Read the model definition and answer for the solid it produces. Units are mm, in the model's axes. Face numbers are marked on the shaded views. Coordinates: 2 decimals unless noted, no trailing zeros. One line per item, written item: value. Start each with the question number.
1. For a pull along X with two mould halves and no side action, classify the marked faces 1 and 2 as pulls with the +X half, pulls with the -X half, needs draft (parallel to the pull), parting line crosses it, or undercut.
2. Given P1, Ø1, axis at x = -81.5, y = 5.5, coming from the -Z side; P2, Ø5, axis at x = -4.5, y = 31, coming from the +Z side; P3, Ø4, axis at y = 23, z = 21.5, coming from the -X side; P4, Ø15.5, axis at x = -4.5, z = -5, coming from the +Y side, each flat-ended and moving along its own axis, determine where each tip first touches the part or whether it passes through.
3. Consider line 1 along X through (y, z) = (19.5, 0); line 2 along Z through (x, y) = (1.5, 19); line 3 along Y through (x, z) = (90.5, 48.5). Determine where each line is inside the solid, lowest interval first.
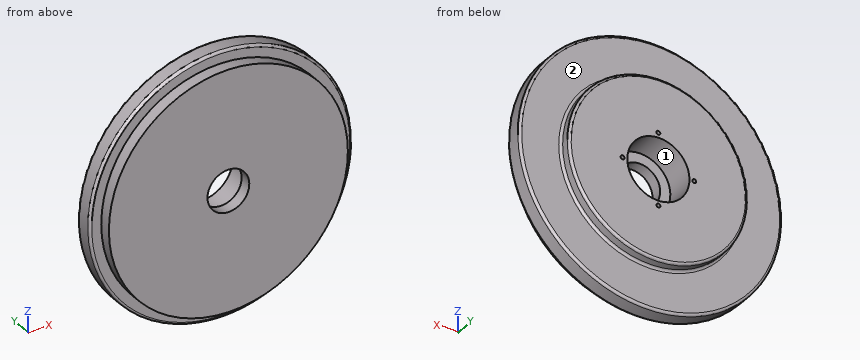
```python
from build123d import *

# Parameters (mm, degrees)
SKETCH1_R           = 100
BOSS_EXTRUDE1_DEPTH = 10
SKETCH2_R           = 110
BOSS_EXTRUDE2_DEPTH = 15
SKETCH3_R           = 75
BOSS_EXTRUDE3_DEPTH = 10
FILLET1_R           = 2
SKETCH4_R           = 26
CUT_EXTRUDE1_DEPTH  = 25
SKETCH5_R           = 17.5
CUT_EXTRUDE2_DEPTH  = 158.559512566
CIRPATTERN1_COUNT   = 4
FILLET2_R           = 2


with BuildPart() as part:
    # Sketch1 → Boss-Extrude1 (new body)
    with BuildSketch(Plane(origin=(0, 0, 0), x_dir=(1, 0, 0), z_dir=(0, 1, 0))):
        with Locations(Location((0, 0, 0), (0, 0, 270))):
            Circle(SKETCH1_R)
    extrude(amount=BOSS_EXTRUDE1_DEPTH)

    # Sketch2 → Boss-Extrude2 (add)
    with BuildSketch(Plane(origin=(0, 10, 0), x_dir=(1, 0, 0), z_dir=(0, 1, 0))):
        with Locations(Location((0, 0, 0), (0, 0, 270))):
            Circle(SKETCH2_R)
    extrude(amount=BOSS_EXTRUDE2_DEPTH)

    # Sketch3 → Boss-Extrude3 (add)
    with BuildSketch(Plane(origin=(0, 25, 0), x_dir=(1, 0, 0), z_dir=(0, 1, 0))):
        with Locations(Location((0, 0, 0), (0, 0, 270))):
            Circle(SKETCH3_R)
    extrude(amount=BOSS_EXTRUDE3_DEPTH)

    # Fillet1
    fillet1_edges = [part.edges().sort_by_distance(p)[0] for p in [
        (0, 25, -75),
        (0, 35, -75),
    ]]
    fillet(fillet1_edges, radius=FILLET1_R)

    # Sketch4 → Cut-Extrude1 (cut)
    with BuildSketch(Plane(origin=(0, 35, 0), x_dir=(1, 0, 0), z_dir=(0, 1, 0))):
        with Locations(Location((0, 0, 0), (0, 0, 270))):
            Circle(SKETCH4_R)
    extrude(amount=-CUT_EXTRUDE1_DEPTH, mode=Mode.SUBTRACT)

    # Sketch5 → Cut-Extrude2 (cut, through all)
    with BuildSketch(Plane(origin=(0, 10, 0), x_dir=(1, 0, 0), z_dir=(0, 1, 0))):
        with Locations(Location((0, 0, 0), (0, 0, 270))):
            Circle(SKETCH5_R)
    extrude(amount=-CUT_EXTRUDE2_DEPTH, mode=Mode.SUBTRACT)

    # Sketch8 → M4 Tapped Hole1 (revolve, cut)
    with BuildSketch(Plane(origin=(0, 35, -30), x_dir=(0, 0, 1), z_dir=(1, 0, 0))):
        Polygon((0, 0), (0, 11.091420021), (1.65, 10.1), (1.65, 0), align=None)
    m4_tapped_hole1 = revolve(axis=Axis((0, 41.35, -30), (0, -1, 0)), mode=Mode.SUBTRACT)

    # CirPattern1: M4 Tapped Hole1 ×4 about axis
    cirpattern1_axis = Axis((0, 0, 0), (0, 1, 0))
    for i in range(1, CIRPATTERN1_COUNT):
        add(m4_tapped_hole1.rotate(cirpattern1_axis, i * 360 / CIRPATTERN1_COUNT), mode=Mode.SUBTRACT)

    # Fillet2
    fillet2_edges = [part.edges().sort_by_distance(p)[0] for p in [
        (0, 10, -110),
        (0, 25, -110),
    ]]
    fillet(fillet2_edges, radius=FILLET2_R)


solid = part.part
```
Answer block:
1. face 1: undercut
1. face 2: needs draft
2. P1: stops at z = -58.64
2. P2: stops at z = 74.97
2. P3: stops at x = -108.26
2. P4: passes through
3. line 1: x = -110 to -26, 26 to 110
3. line 2: z = -109.99 to -25.96, 25.96 to 109.99
3. line 3: y = 10 to 25
